```python
from build123d import *

# Parameters (mm, degrees)
M22X1_5_1_D         = 20.5
SKETCH_4_OUTSIDE_W  = 49.818
SKETCH_4_OUTSIDE_H  = 49.818
CUT_EXTRUDE_1_DEPTH = 18


with BuildPart() as part:
    # 草图1 → 旋转1 (revolve)
    with BuildSketch(Plane.XY, mode=Mode.PRIVATE) as revolve_1_sk:
        with BuildLine():
            Line((-18, 7.77364393), (-18, 30))
            Line((-18, 30), (-10, 30))
            Line((-10, 30), (-10, 5.2))
            Line((-10, 5.2), (-11.25, 4))
            Line((-11.25, 4), (-11.25, 0))
            Line((-11.25, 0), (-13, 0))
            ThreePointArc((-13, 0), (-15.979905663, 3.578147123), (-18, 7.77364393))
        make_face()
    revolve(revolve_1_sk.sketch.rotate(Axis((0, 29.86875, 0), (0, -1, 0)), 270), axis=Axis((0, 29.86875, 0), (0, -1, 0)))

    # M22x1.5 螺纹孔1 (through all)
    with Locations(Plane(origin=(0, 30, 0), x_dir=(1, 0, 0), z_dir=(0, 1, 0))):
        with Locations((0, 0)):
            Hole(M22X1_5_1_D / 2)

    # 草图4 outside → 切除-拉伸1 (cut)
    with BuildSketch(Plane(origin=(0, 30, 0), x_dir=(1, 0, 0), z_dir=(0, 1, 0))):
        Rectangle(SKETCH_4_OUTSIDE_W, SKETCH_4_OUTSIDE_H)
        Polygon((-8.65, 15), (8.65, 15), (17.3, 0), (8.65, -15), (-8.65, -15), (-17.3, 0), align=None, mode=Mode.SUBTRACT)
    extrude(amount=-CUT_EXTRUDE_1_DEPTH, mode=Mode.SUBTRACT)

    # 草图6 → 切除-旋转8 (revolve, cut)
    with BuildSketch(Plane(origin=(0, 0, 0), x_dir=(0, 0, -1), z_dir=(1, 0, 0)), mode=Mode.PRIVATE) as cut_revolve_8_sk:
        Polygon((6.162949371, 32.348642693), (24.147556169, 27.529681825), (24.147556169, 34), (6.162949371, 34), align=None)
    revolve(cut_revolve_8_sk.sketch.rotate(Axis((0, 32.348642693, 0), (0, 1, 0)), 90), axis=Axis((0, 32.348642693, 0), (0, 1, 0)), mode=Mode.SUBTRACT)


solid = part.part
```
Source: CAD feature listing. Evaluate the final solid. Frame: model axes, mm. A direction names the side the tool comes from. Give positions to 0.01 mm unless a question says otherwise; leave off trailing zeros. Loops run counter-clockwise (first coordinate to the right, second up) from the corner with the lowest first, then second, coordinate; pieces in that order, holes last. Notation, with made-up numbers: (57, 58) -> (99, 58) arc R18 cw to (99, 74) -> close; hole circle Ø2 at (79.5, 52.5). An arc over 180 degrees is marked (long way). Use a Markdown table: item, result. Add a question column.
(1) First-contact query: pin 1 Ø1 at (x, y) = (13, 22) entering from -Z; pin 2 Ø1 at (x, y) = (-10.5, 21) entering from -Z; pin 3 Ø3 at (y, z) = (18, -9.5) entering from +X; pin 4 Ø18.5 at (x, z) = (0, 0) entering from +Y. Flat tips, straight axial feed; report the tip coordinate or a pass-through.
(2) Section query C-C (y = 6.25). Output: boundary loops of the cut face in (x, z).
(3) Section query B-B (x = 0). Output: boundary loops of the cut face in (y, z), then the cut area to 3 significant figures.
(4) Access query for faces 4 (the face through (0, 21, 15)), 5 (the face through (4.31, 1.97, 10.39)), 6 (the face through (12.914, 21.118, -7.605)), 7 (the face through (-13, 12, 8)). Directions: +Z, -Z, +X, -X, +Y, -Y. A direction counts if a zero-diameter tool reaches every point of the face in a straight line with its end or side. Return the directions, or none.
(5) Section query A-A (y = 13.75). Output: boundary loops of the cut face in (x, z), then the cut area to 3 significant figures.
(6) Ray query, line 1 (Z direction, x = 0, y = 21); line 2 (Z direction, x = -7, y = 3.5); line 3 (X direction, y = 11.75, z = -0.5). Return the intervals inside material, ascending.
(7) Pull-direction query (X, two-part tool) for faces 1 (the face through (13.036, 21.118, 7.395)), 2 (the face through (-5.407, 9.916, 17.169)), 3 (the face through (2.222, 17.305, 10.006)); classes: +X half, -X half, draft (parallel to the pull), parting line (faces both ways), or undercut.
Checked values:
| question | item | result |
|---|---|---|
| 1 | pin 1 | z = -8.32 |
| 1 | pin 2 | z = -12.66 |
| 1 | pin 3 | x = 12.69 |
| 1 | pin 4 | through |
| 2 | outline | circle Ø34.82 at (0, 0); hole circle Ø20.5 at (0, 0) |
| 3 | outline | (0, -13) arc R19 ccw to (7.77, -18) -> (12, -18) -> (12, -15) -> (29.98, -15) -> (30, -14.93) -> (30, -10.25) -> (4.96, -10.25) -> (4, -11.25) -> (0, -11.25) -> close; (0, 11.25) -> (4, 11.25) -> (4.96, 10.25) -> (30, 10.25) -> (30, 14.93) -> (29.98, 15) -> (12, 15) -> (12, 18) -> (7.77, 18) arc R19 ccw to (0, 13) -> close |
| 3 | area | 316 mm^2 |
| 4 | face 4 | +Z, +X, -X, +Y |
| 4 | face 5 | -Y |
| 4 | face 6 | -Z, +X, +Y |
| 4 | face 7 | +Y |
| 5 | outline | (-17.3, 0) -> (-8.65, -15) -> (8.65, -15) -> (17.3, 0) -> (8.65, 15) -> (-8.65, 15) -> close; hole circle Ø20.5 at (0, 0) |
| 5 | area | 448 mm^2 |
| 6 | line 1 | -15 to -10.25, 10.25 to 15 |
| 6 | line 2 | -14.31 to -8.81, 8.81 to 14.31 |
| 6 | line 3 | -17.99 to -10.24, 10.24 to 17.99 |
| 7 | face 1 | +X half |
| 7 | face 2 | parting line |
| 7 | face 3 | undercut |
